from build123d import *

# Parameters (mm, degrees)
SKETCH_1_W          = 12
SKETCH_1_H          = 40
SKETCH_1_R          = 3.5
EXTRUDE_1_DEPTH     = 6
CUT_EXTRUDE_1_REACH = 26.083
SKETCH_2_R          = 3.5


with BuildPart() as part:
    # 草图1 → 凸台-拉伸1 (new, symmetric)
    with BuildSketch(Plane.XY):
        Rectangle(SKETCH_1_W, SKETCH_1_H)
        with Locations((0, 14)):
            Circle(SKETCH_1_R, mode=Mode.SUBTRACT)
        with Locations((0, -14)):
            Circle(SKETCH_1_R, mode=Mode.SUBTRACT)
    extrude(amount=EXTRUDE_1_DEPTH, both=True)

    # 草图2 → 切除-拉伸1 (cut, up to next)
    with BuildSketch(Plane(origin=(6, 0, 0), x_dir=(0, 0, -1), z_dir=(1, 0, 0)), mode=Mode.PRIVATE) as cut_extrude_1_sk1:
        Circle(SKETCH_2_R)
    cut_extrude_1_tool1 = extrude(cut_extrude_1_sk1.sketch, amount=-CUT_EXTRUDE_1_REACH, mode=Mode.PRIVATE) & part.part
    add(cut_extrude_1_tool1.solids().sort_by_distance((6, 0, 0))[0], mode=Mode.SUBTRACT)


solid = part.part
Input: part model. Units: mm. Frame: model coordinates. Coordinates: 2 decimals unless noted, no trailing zeros. Loops run counter-clockwise (first coordinate to the right, second up) from the corner with the lowest first, then second, coordinate; pieces in that order, holes last.
Q1. Cut plane D-D (x = -2). Output: boundary loops of the cut face in (y, z).
Q2. Cut plane A-A (z = 0). Output: boundary loops of the cut face in (x, y), then the cut area to 3 significant figures.
Q3. Draft query along X for faces 1 (the face through (-6, 0, 4)), 2 (the face through (-0.759, -17.417, -0.084)), 3 (the face through (0, 0, -6)). Return one class per face: +X half, -X half, draft (parallel to the pull), parting line (faces both ways), or undercut.
Q4. Cut plane C-C (y = 0). Output: boundary loops of the cut face in (x, z), then the cut area to 3 significant figures.
Q5. Material intervals for line 1 (Y direction, x = -1, z = -1.5); line 2 (Y direction, x = 0.5, z = -2.75); line 3 (X direction, y = 13, z = -0.25), sorted ascending.
Q6. Cut plane B-B (x = 0). Output: boundary loops of the cut face in (y, z), then the cut area to 3 significant figures.
Working result:
1. outline: (-20, -6) - (-16.87, -6) - (-16.87, 6) - (-20, 6) - close; (-11.13, -6) - (11.13, -6) - (11.13, 6) - (-11.13, 6) - close; (16.87, -6) - (20, -6) - (20, 6) - (16.87, 6) - close; hole circle Ø7 at (0, 0)
2. outline: (-6, -20) - (6, -20) - (6, -3.5) - (-6, -3.5) - close; (-6, 3.5) - (6, 3.5) - (6, 20) - (-6, 20) - close; hole circle Ø7 at (0, -14); hole circle Ø7 at (0, 14)
2. area: 319 mm2
3. face 1: -X half
3. face 2: undercut
3. face 3: draft
4. outline: (-6, -6) - (6, -6) - (6, -3.5) - (-6, -3.5) - close; (-6, 3.5) - (6, 3.5) - (6, 6) - (-6, 6) - close
4. area: 60.0 mm2
5. line 1: y = -20 to -17.35, -10.65 to -3.16, 3.16 to 10.65, 17.35 to 20
5. line 2: y = -20 to -17.46, -10.54 to -2.17, 2.17 to 10.54, 17.46 to 20
5. line 3: x = -6 to -3.35, 3.35 to 6
6. outline: (-20, -6) - (-17.5, -6) - (-17.5, 6) - (-20, 6) - close; (-10.5, -6) - (10.5, -6) - (10.5, 6) - (-10.5, 6) - close; (17.5, -6) - (20, -6) - (20, 6) - (17.5, 6) - close; hole circle Ø7 at (0, 0)
6. area: 274 mm2
